from build123d import *

# Parameters (mm, degrees)
HEX_HEAD_DEPTH                 = 4
HEAD_CHAMFER_PROFILE_OUTSIDE_W = 23.158
HEAD_CHAMFER_PROFILE_OUTSIDE_H = 24.706
HEAD_CHAMFER_PROFILE_OUTSIDE_R = 5
HEAD_CHAMFER_45DEG_DEPTH       = 4
HEAD_CHAMFER_45DEG_DRAFT       = -45
SHANK_PROFILE_5_R              = 2.5
SHANK_5X9_DEPTH                = 9


with BuildPart() as part:
    # Hex Head Profile → Hex Head (new body)
    with BuildSketch(Plane.XY):
        Polygon((5, -2.886751346), (5, 2.886751346), (0, 5.773502692), (-5, 2.886751346), (-5, -2.886751346), (0, -5.773502692), align=None)
    extrude(amount=HEX_HEAD_DEPTH)


with BuildPart() as head_chamfer_45deg_tool:
    # Head Chamfer Profile outside → Head Chamfer 45deg (with draft: the straight prism first)
    with BuildSketch(Plane.XY.offset(4)):
        Rectangle(HEAD_CHAMFER_PROFILE_OUTSIDE_W, HEAD_CHAMFER_PROFILE_OUTSIDE_H)
        Circle(HEAD_CHAMFER_PROFILE_OUTSIDE_R, mode=Mode.SUBTRACT)
    extrude(amount=-HEAD_CHAMFER_45DEG_DEPTH)
    # Head Chamfer 45deg: the draft: its side faces are tilted about the plane it starts from
    head_chamfer_45deg_sides = [head_chamfer_45deg_tool.faces().sort_by_distance(p)[0] for p in [
        (0, -12.353, 2),
        (11.579, 0, 2),
        (0, 12.353, 2),
        (-11.579, 0, 2),
        (-5, 0, 2),
    ]]
    draft(head_chamfer_45deg_sides, Plane.XY.offset(4), HEAD_CHAMFER_45DEG_DRAFT)


with BuildPart() as part_1:
    add(part.part)

    # Head Chamfer 45deg: cut by head_chamfer_45deg_tool
    add(head_chamfer_45deg_tool.part, mode=Mode.SUBTRACT)

    # Shank Profile Ø5 → Shank Ø5x9 (add)
    with BuildSketch(Plane(origin=(0, 0, 0), x_dir=(-1, 0, 0), z_dir=(0, 0, -1))):
        Circle(SHANK_PROFILE_5_R)
    extrude(amount=SHANK_5X9_DEPTH)


solid = part_1.part
Source: CAD feature listing. Evaluate the final solid. Frame: model axes, mm. A direction names the side the tool comes from. Coordinates: 2 decimals unless noted, no trailing zeros. Order: outer loops, then holes, each group sorted by start corner. A loop starts at its lowest first (then second) coordinate and runs counter-clockwise, first axis right, second up. Notation, with made-up numbers: M 13.5,-10 L 70.5,-10 A6 ccw 70.5,-5 Z; hole C -14.75,7 d7. An arc over 180 degrees is marked long. Write each question's results on one line, items separated by ' | '. Start each with the question number.
1. Reachability of faces 1 (the face through (2.465, -4.35, 1.972)), 2 (the face through (-1.2, -2.5, 0)) from +Z, -Z, +X, -X, +Y, -Y: full face, straight path, thin tool, end or side. Return the list, or none.
2. Material intervals for L1, parallel to Z at x = 0.75, y = -3.25; L2, parallel to Y at x = 2.5, z = 1.5; L3, parallel to Y at x = 1.5, z = 3, sorted ascending.
3. Section A-A, the plane z = 2. Return the cut outline in (x, y), then the cut area to 3 significant figures.
4. Pin query (flat end, axial travel): pin 1 (1 mm diameter, centred on x = -2, y = -4.5, fed in from -Z); pin 2 (3 mm diameter, centred on x = -2.5, z = 0, fed in from -Y); pin 3 (5 mm diameter, centred on x = 3.5, z = -7.5, fed in from -Y). Return the tip coordinate at first contact, or that it passes through.
5. Section B-B, the plane z = -7.25. Return the cut outline in (x, y).
Solution:
1) face 1: +Z, -Z, +X, -Y | face 2: -Z
2) L1: 0 to 4 | L2: -4.33 to 4.33 | L3: -4.91 to 4.91
3) outline: M -5,-2.89 L 0,-5.77 L 5,-2.89 L 5,2.89 L 0,5.77 L -5,2.89 Z | area: 86.6 mm²
4) pin 1: z = 0 | pin 2: y = -5.2 | pin 3: y = -2.29
5) outline: C 0,0 d5
